Geometry check sheet. Reference: the model listing, model coordinates, mm. A direction names the side the tool comes from. Coordinates: 2 decimals unless noted, no trailing zeros. Write each loop counter-clockwise with the first axis right and the second up, starting at its lowest first coordinate (ties: lowest second). Pieces come first, ordered by that corner, then holes. Notation, with made-up numbers: M 8,77 L 62,77 A33 ccw 62,107 Z; hole C 16,18.5 d7. An arc over 180 degrees is marked long. Put each result on its own line as item: value. Start each with the question number.
1) Cross-section at D-D on z = 1.25. Record the cut outline in (x, y).
2) Set-up check for faces 5 (the cylindrical face through (-8.74, 5.71, 11.04)), 6 (the flat face through (4.42, 0.35, 7.4)), 7 (the flat face through (-12.036, -2.8, 14.5)): record each of +Z, -Z, +X, -X, +Y, -Y from which the full face is reachable in a straight line by a thin tool's end or side.
3) Mould release check, pull along Y, two halves, no side actions. Record for faces 1 (the cylindrical face through (-8.022, -11.638, 4.262)), 2 (the flat face through (-5.236, -2.8, 14.5)), 3 (the flat face through (-17.667, 0, 7.395)), 4 (the cylindrical face through (-8.81, -10.863, 12.638)): released by +Y, released by -Y, zero draft, split by the parting line, or undercut.
4) Cross-section at C-C on z = 6.25. Record the cut outline in (x, y).
5) Cross-section at B-B on y = 2. Record the cut outline in (x, z).
6) Scan lines: line 1 along Z through (x, y) = (-14.75, -7); line 2 along Y through (x, z) = (-8, 10.5); line 3 along Z through (x, y) = (-7.25, 3.75). Record each from-to range of solid material in increasing order.
7) Cross-section at A-A on z = 3.75. Record the cut outline in (x, y).
8) Gauge pin test, flat ends, axial feed: pin 1 (5 mm diameter, centred on y = -0.5, z = 10.5, fed in from +X); pin 2 (0.5 mm diameter, centred on y = -2, z = 14.5, fed in from +X); pin 3 (5 mm diameter, centred on y = -6, z = 2, fed in from -X). Record the tip position at first contact, or that the pin passes through.
from build123d import *

# Parameters (mm, degrees)
SKETCH_1_W          = 25.3
SKETCH_1_H          = 24.8
EXTRUDE_1_DEPTH     = 15
CUT_EXTRUDE_1_REACH = 30.897
CUT_EXTRUDE_2_REACH = 37.009
SKETCH_3_W          = 6.8
SKETCH_3_H          = 1
CUT_EXTRUDE_3_REACH = 33.713
SKETCH_5_R          = 4.5
SKETCH_7_R          = 0.8
CUT_EXTRUDE_4_DEPTH = 6


with BuildPart() as part:
    # 草图1 → 凸台-拉伸1 (new body)
    with BuildSketch(Plane.XY):
        with Locations((-6.986164384, -2.581917808)):
            Rectangle(SKETCH_1_W, SKETCH_1_H)
    extrude(amount=EXTRUDE_1_DEPTH)

    # 草图2 → 切除-拉伸1 (cut, up to next)
    with BuildSketch(Plane(origin=(0, 0, 0), x_dir=(-1, 0, 0), z_dir=(0, 0, -1)), mode=Mode.PRIVATE) as cut_extrude_1_sk1:
        Polygon((-5.663835616, 9.818082192), (-2.403835616, -14.981917808), (-5.663835616, -14.981917808), align=None)
    cut_extrude_1_tool1 = extrude(cut_extrude_1_sk1.sketch, amount=-CUT_EXTRUDE_1_REACH, mode=Mode.PRIVATE) & part.part
    # 草图2 → 切除-拉伸1 (cut, up to next)
    with BuildSketch(Plane(origin=(0, 0, 0), x_dir=(-1, 0, 0), z_dir=(0, 0, -1)), mode=Mode.PRIVATE) as cut_extrude_1_sk2:
        Polygon((16.376164384, 9.818082192), (19.636164384, 9.818082192), (19.636164384, -14.981917808), align=None)
    cut_extrude_1_tool2 = extrude(cut_extrude_1_sk2.sketch, amount=-CUT_EXTRUDE_1_REACH, mode=Mode.PRIVATE) & part.part
    add(cut_extrude_1_tool1.solids().sort_by_distance((4.577169, -6.715251, 0))[0], mode=Mode.SUBTRACT)
    add(cut_extrude_1_tool2.solids().sort_by_distance((-18.549498, 1.551416, 0))[0], mode=Mode.SUBTRACT)

    # 草图3 → 切除-拉伸2 (cut, up to next)
    with BuildSketch(Plane.XZ.offset(14.981917808), mode=Mode.PRIVATE) as cut_extrude_2_sk1:
        with Locations((-8.636164384, 14.5)):
            Rectangle(SKETCH_3_W, SKETCH_3_H)
    cut_extrude_2_tool1 = extrude(cut_extrude_2_sk1.sketch, amount=-CUT_EXTRUDE_2_REACH, mode=Mode.PRIVATE) & part.part
    add(cut_extrude_2_tool1.solids().sort_by_distance((-8.636164, -14.981918, 14.5))[0], mode=Mode.SUBTRACT)

    # 草图5 → 切除-拉伸3 (cut, up to next)
    with BuildSketch(Plane(origin=(4.298949072, -0.565103789, 0), x_dir=(0, 0, -1), z_dir=(0.9914706167018176, -0.13033041171160964, 0)), mode=Mode.PRIVATE) as cut_extrude_3_sk1:
        with Locations(Location((-7, -9.013320677, 0), (0, 0, 90))):
            Circle(SKETCH_5_R)
    cut_extrude_3_tool1 = extrude(cut_extrude_3_sk1.sketch, amount=-CUT_EXTRUDE_3_REACH, mode=Mode.PRIVATE) & part.part
    add(cut_extrude_3_tool1.solids().sort_by_distance((3.124239, -9.501546, 7))[0], mode=Mode.SUBTRACT)

    # 草图7 → 切除-拉伸4 (cut)
    with BuildSketch(Plane.XY.offset(14)):
        with Locations((-8.636164384, 4.918082192)):
            Circle(SKETCH_7_R)
        with Locations((-8.636164384, -10.081917808)):
            Circle(SKETCH_7_R)
    extrude(amount=-CUT_EXTRUDE_4_DEPTH, mode=Mode.SUBTRACT)


solid = part.part
Answer key:
1. outline: M -19.64,-14.98 L 2.4,-14.98 L 5.66,9.82 L -16.38,9.82 Z
2. face 5: +Z
2. face 6: +Z, -Z, +X, -Y
2. face 7: +Z, +Y, -Y
3. face 1: undercut
3. face 2: zero draft
3. face 3: released by +Y
3. face 4: undercut
4. outline: M -19.64,-14.98 L 2.4,-14.98 L 2.55,-13.9 L -19.12,-11.05 Z; M -17.96,-2.25 L 3.7,-5.1 L 5.66,9.82 L -16.38,9.82 Z
5. outline: M -17.4,0 L 4.64,0 L 4.64,15 L -5.24,15 L -5.24,14 L -12.04,14 L -12.04,15 L -17.4,15 Z
6. line 1: z = 0 to 2.5, 11.5 to 15
6. line 2: y = -14.98 to -10.89, -5.19 to 4.43, 5.4 to 9.82
6. line 3: z = 0 to 14
7. outline: M -19.64,-14.98 L 2.4,-14.98 L 2.72,-12.59 L -18.95,-9.74 Z; M -18.14,-3.57 L 3.53,-6.42 L 5.66,9.82 L -16.38,9.82 Z
8. pin 1: stops at x = 4.64
8. pin 2: stops at x = 4.14
8. pin 3: stops at x = -18.78
